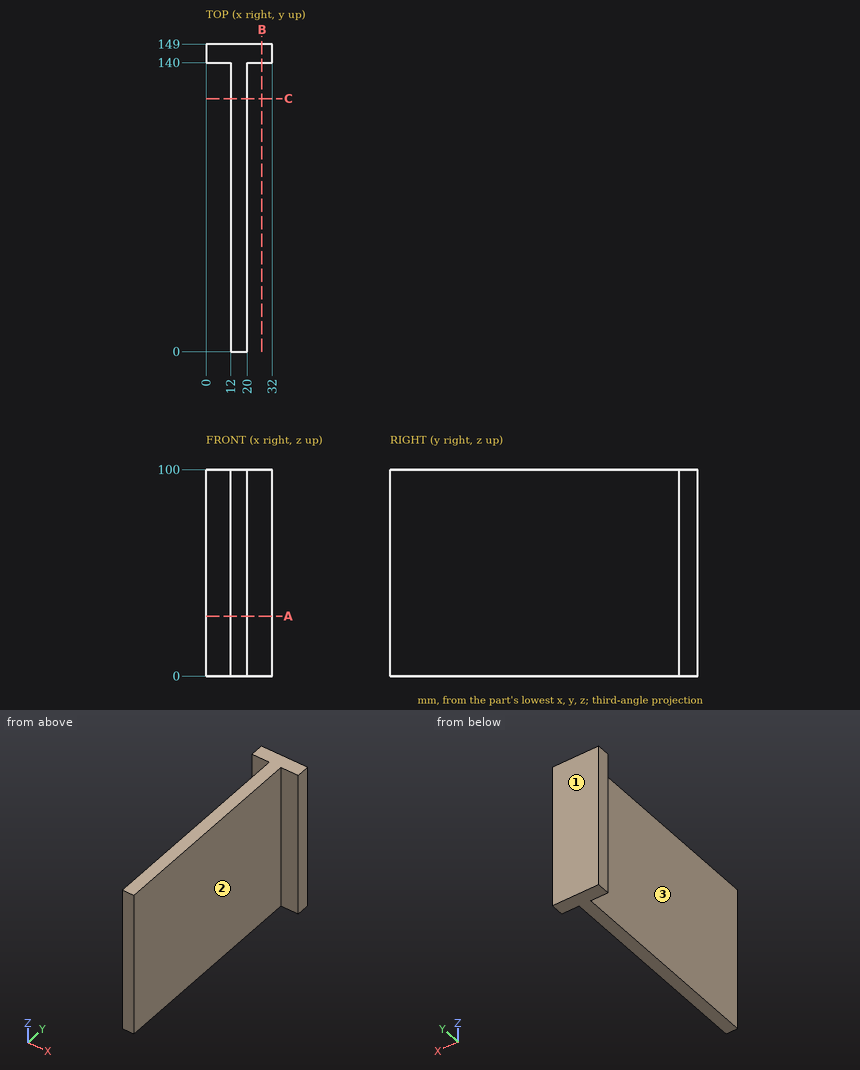
Geometry: see drawing. Coordinates: mm, zero at the bounding-box minimum. Give positions to 0.01 mm unless a question says otherwise; leave off trailing zeros. Loops run counter-clockwise (first coordinate to the right, second up) from the corner with the lowest first, then second, coordinate; pieces in that order, holes last. Notation, with made-up numbers: (-11.75, -19) - (1.25, -19) arc R7 ccw to (1.25, -6) - close; hole circle Ø11 at (75, -3). An arc over 180 degrees is marked (long way). Use CSV: the item, a comma, the result in double quotes. Start each with the question number.
1. Pin query (flat end, axial travel): pin 1 (5 mm diameter, centred on y = 45.5, z = 35, fed in from -X); pin 2 (10 mm diameter, centred on x = 20, z = 29.5, fed in from -Y); pin 3 (1.5 mm diameter, centred on y = 68, z = 31.5, fed in from +X); pin 4 (6 mm diameter, centred on x = 28, z = 45.5, fed in from -Y). Return the tip coordinate at first contact, or that it passes through.
2. Section C-C (y = 122.5). Output: boundary loops of the cut face in (x, z).
3. Ray query, L1, parallel to Y at x = 22, z = 50.5; L2, parallel to X at y = 79.5, z = 20. Return the intervals inside material, ascending.
4. Section B-B (x = 27). Output: boundary loops of the cut face in (y, z).
5. Draft query along X for the marked faces 1, 2 and 3. Return one class per face: +X half, -X half, draft (parallel to the pull), parting line (faces both ways), or undercut.
6. Section A-A (z = 29). Output: boundary loops of the cut face in (x, y), then the cut area to 3 significant figures.
Response:
1,pin 1,"x = 12"
1,pin 2,"y = 0"
1,pin 3,"x = 20"
1,pin 4,"y = 140"
2,outline,"(12, 0) - (20, 0) - (20, 100) - (12, 100) - close"
3,L1,"140 to 149"
3,L2,"12 to 20"
4,outline,"(140, 0) - (149, 0) - (149, 100) - (140, 100) - close"
5,face 1,"draft"
5,face 2,"+X half"
5,face 3,"-X half"
6,outline,"(0, 140) - (12, 140) - (12, 0) - (20, 0) - (20, 140) - (32, 140) - (32, 149) - (0, 149) - close"
6,area,"1,410 mm²"
